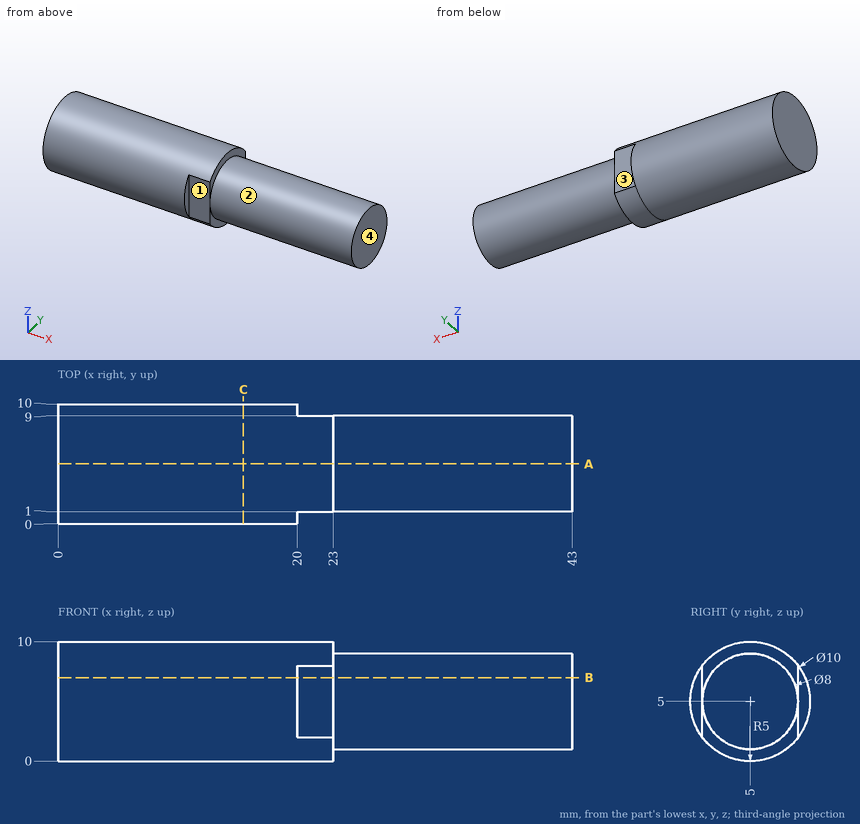
Input: dimensioned drawing with shaded views. Units: mm. Origin: part minimum x, y, z. A direction names the side the tool comes from. Coordinates: 2 decimals unless noted, no trailing zeros. Loops run counter-clockwise (first coordinate to the right, second up) from the corner with the lowest first, then second, coordinate; pieces in that order, holes last. Notation, with made-up numbers: (-18, 70) -> (5, 70) arc R29 ccw to (5, 106) -> close; hole circle Ø7 at (83, 60). An arc over 180 degrees is marked (long way). One line per item, written item: value. Start each with the question number.
Q1. Section query C-C, the plane x = 15.5. Return the cut outline in (y, z).
Q2. Set-up query: the marked faces 1, 2, 3 and 4. Return all of +Z, -Z, +X, -X, +Y, -Y with unobstructed straight access to the full face (end or side cutting, diameter ignored); none if empty.
Q3. Section query A-A, the plane y = 5. Return the cut outline in (x, z).
Q4. Contact query for flat-ended pins moving along their axis: P1, Ø3, axis at x = 37, z = 2, coming from the +Y side; P2, Ø3, axis at x = 30, y = 7.5, coming from the -Z side; P3, Ø1.5, axis at x = 21.5, z = 5.5, coming from the +Y side. Output: stop coordinate, or through.
Q5. Section query B-B, the plane z = 7. Return the cut outline in (x, y).
Q6. Line query: line 1 along X through (y, z) = (2.5, 0.75); line 2 along Z through (x, y) = (26, 4.75); line 3 along X through (y, z) = (0.5, 4.5). Output: solid intervals per line, ascending.
Results:
1. outline: circle Ø10 at (5, 5)
2. face 1: +Z, -Z, +X, -Y
2. face 2: +X
2. face 3: +Z, -Z, +X, +Y
2. face 4: +Z, -Z, +X, +Y, -Y
3. outline: (0, 0) -> (23, 0) -> (23, 1) -> (43, 1) -> (43, 9) -> (23, 9) -> (23, 10) -> (0, 10) -> close
4. P1: y = 8.71
4. P2: z = 1.13
4. P3: y = 9
5. outline: (0, 0.42) -> (20, 0.42) -> (20, 1) -> (23, 1) -> (23, 1.54) -> (43, 1.54) -> (43, 8.46) -> (23, 8.46) -> (23, 9) -> (20, 9) -> (20, 9.58) -> (0, 9.58) -> close
6. line 1: 0 to 23
6. line 2: 1.01 to 8.99
6. line 3: 0 to 20
